Job drawing, mm, ordinate dimensions from the low corner. One solid piece. Give positions to 0.01 mm unless a question says otherwise; leave off trailing zeros. Write each loop counter-clockwise with the first axis right and the second up, starting at its lowest first coordinate (ties: lowest second). Pieces come first, ordered by that corner, then holes. Notation, with made-up numbers: (70.25, 6.5) - (97.25, 6.5) arc R25 ccw to (97.25, 41.5) - close; hole circle Ø9 at (86.25, -6). An arc over 180 degrees is marked (long way). Answer as a JSON object with one key per item and string values.
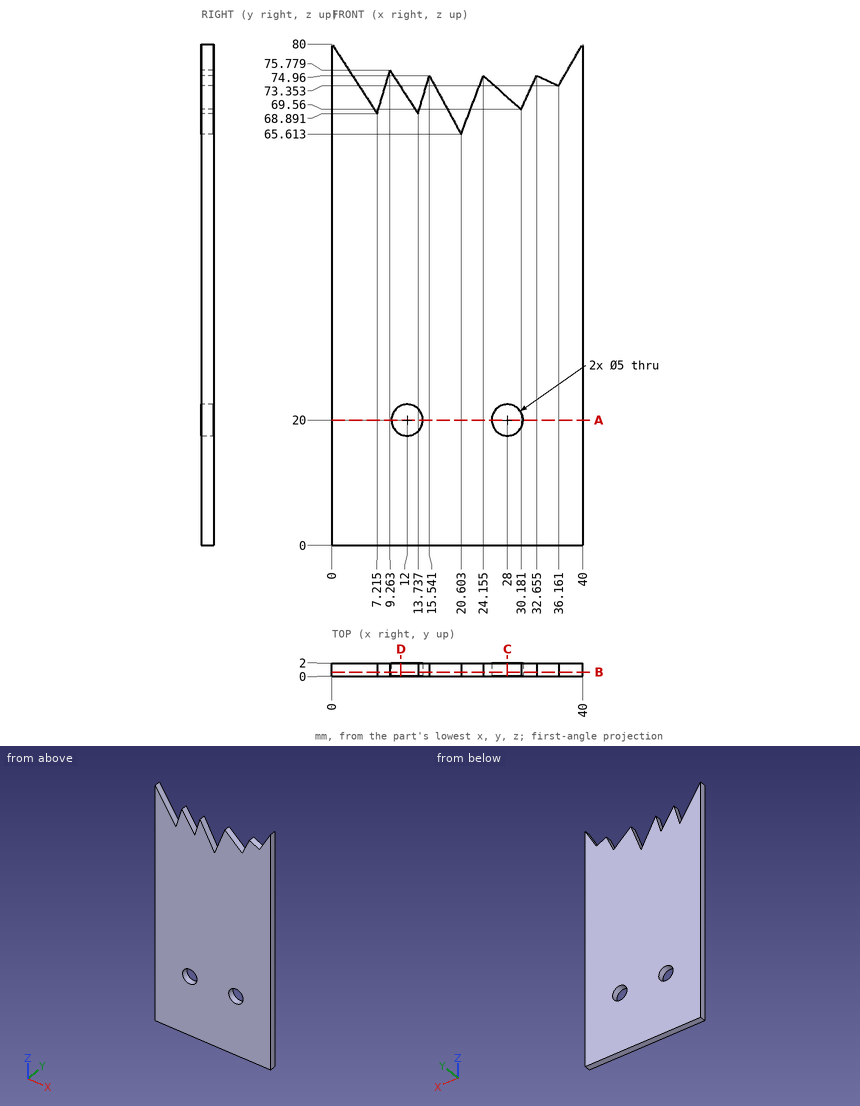
Item 1: Cut at C-C (x = 28). Give the cut face in (y, z) (1 decimal), and give its area (3 significant figures).
Entries:
{"outline": "(0, 0) - (2, 0) - (2, 17.5) - (0, 17.5) - close; (0, 22.5) - (2, 22.5) - (2, 71.5) - (0, 71.5) - close", "area": "133 mm2"}
Item 2: Cut at A-A (z = 20). Give the cut face in (x, y).
Entries:
{"outline": "(0, 0) - (9.5, 0) - (9.5, 2) - (0, 2) - close; (14.5, 0) - (25.5, 0) - (25.5, 2) - (14.5, 2) - close; (30.5, 0) - (40, 0) - (40, 2) - (30.5, 2) - close"}
Item 3: Cut at D-D (x = 11). Give the cut face in (y, z) (1 decimal).
Entries:
{"outline": "(0, 0) - (2, 0) - (2, 17.7) - (0, 17.7) - close; (0, 22.3) - (2, 22.3) - (2, 73.1) - (0, 73.1) - close"}
Item 4: Cut at B-B (y = 0.6). Give the cut face in (x, z) (1 decimal), and give its area (3 significant figures).
Entries:
{"outline": "(0, 0) - (40, 0) - (40, 80) - (36.2, 73.4) - (32.7, 75) - (30.2, 69.6) - (24.2, 75) - (20.6, 65.6) - (15.5, 75) - (13.7, 68.9) - (9.3, 75.8) - (7.2, 68.9) - (0, 80) - close; hole circle Ø5 at (12, 20); hole circle Ø5 at (28, 20)", "area": "2,870 mm2"}
Item 5: Probe line 1 (X direction, y = 1, z = 20); line 2 (Z direction, x = 29.5, y = 0.8); line 3 (Z direction, x = 27.5, y = 0.5). List the from-to ranges inside material, lowest first. Write a range as from..to.
Entries:
{"line 1": "0..9.5, 14.5..25.5, 30.5..40", "line 2": "0..18, 22..70.17", "line 3": "0..17.55, 22.45..71.96"}
Item 6: Flat gauge pin, fed straight in: P1, Ø6, axis at x = 28, z = 20, coming from the +Y side. Where does the tip first touch, or does it go through?
Entries:
{"P1": "y = 2"}
